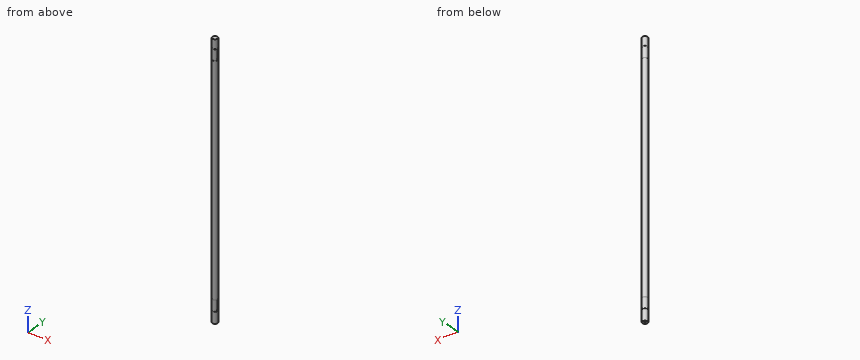
from build123d import *

# Parameters (mm, degrees)
SKETCH_2_R             = 15
EXTRUDE_1_DEPTH        = 1500
CUT_EXTRUDE_1_DEPTH    = 1501.283306579
SKETCH_4_W             = 1.6
SKETCH_4_H             = 0.7
PATTERN_LINEAR_1_COUNT = 2
PATTERN_LINEAR_1_PITCH = 1322
HOLE_WIZARD_M8_1_D     = 6.8
HOLE_WIZARD_M8_1_DEPTH = 19.75
HOLE_WIZARD_M8_1_TIP   = 2.042926105


with BuildPart() as part:
    # 草图2 → 凸台-拉伸1 (new body)
    with BuildSketch(Plane.XY):
        Circle(SKETCH_2_R)
    extrude(amount=EXTRUDE_1_DEPTH)

    # 草图3 → 切除-拉伸1 (cut, through all)
    with BuildSketch(Plane(origin=(10, 0, 0), x_dir=(0, 0, -1), z_dir=(1, 0, 0))):
        with BuildLine():
            Line((-1440, 5), (-1395, 5))
            ThreePointArc((-1395, 5), (-1390, 0), (-1395, -5))
            Line((-1395, -5), (-1440, -5))
            ThreePointArc((-1440, -5), (-1445, 0), (-1440, 5))
        make_face()
        with BuildLine():
            Line((-73, -5), (-118, -5))
            ThreePointArc((-118, -5), (-123, 0), (-118, 5))
            Line((-118, 5), (-73, 5))
            ThreePointArc((-73, 5), (-68, 0), (-73, -5))
        make_face()
    extrude(amount=CUT_EXTRUDE_1_DEPTH, mode=Mode.SUBTRACT)

    # 草图4 → 切除-旋转5 (revolve, cut)
    with BuildSketch(Plane(origin=(0, 0, 0), x_dir=(0, 0, -1), z_dir=(1, 0, 0))):
        with Locations((-1448.3, 14.65)):
            Rectangle(SKETCH_4_W, SKETCH_4_H)
        with Locations((-1386.7, 14.65)):
            Rectangle(SKETCH_4_W, SKETCH_4_H)
    cut_revolve_5 = revolve(axis=Axis((0, 0, 1445), (0, 0, 1)), mode=Mode.SUBTRACT)

    # 阵列(线性)1: 切除-旋转5 ×2
    with Locations(*[(0, 0, -i * PATTERN_LINEAR_1_PITCH) for i in range(1, PATTERN_LINEAR_1_COUNT)]):
        add(cut_revolve_5, mode=Mode.SUBTRACT)

    # M8 螺纹孔1
    with Locations(Plane(origin=(0, 0, 0), x_dir=(-1, 0, 0), z_dir=(0, 0, -1))):
        with Locations((0, 0)):
            Hole(HOLE_WIZARD_M8_1_D / 2, depth=HOLE_WIZARD_M8_1_DEPTH)
            with Locations((0, 0, -(HOLE_WIZARD_M8_1_DEPTH + HOLE_WIZARD_M8_1_TIP / 2))):  # 118° drill point
                Cone(0, HOLE_WIZARD_M8_1_D / 2, HOLE_WIZARD_M8_1_TIP, mode=Mode.SUBTRACT)


solid = part.part
Can you work these out from the model? Positions are in its coordinate system, mm. Give positions to 0.01 mm unless a question says otherwise; leave off trailing zeros. Loops run counter-clockwise (first coordinate to the right, second up) from the corner with the lowest first, then second, coordinate; pieces in that order, holes last. Notation, with made-up numbers: (34, -37) - (78, -37) arc R22 cw to (78, -22) - close; hole circle Ø7 at (53, 78.5). An arc over 180 degrees is marked (long way). Return JSON: item names as keys, results as strings.
1. I want a section at A-A on z = 980.5. Please give me the cut outline in (x, y).
Output values:
{"outline": "circle Ø30 at (0, 0)"}
2. I'm going to push flat-ended pins straight in: pin 1 Ø10 at (x, z) = (3, 572) entering from +Y; pin 2 Ø10 at (x, z) = (12, 508) entering from +Y; pin 3 Ø3 at (x, z) = (5, 1209) entering from -Y; pin 4 Ø4 at (y, z) = (6.5, 412) entering from +X. Where does each tip first touch, or does it pass through?
Output values:
{"pin 1": "stops at y = 15", "pin 2": "stops at y = 13.27", "pin 3": "stops at y = -14.59", "pin 4": "stops at x = 14.31"}
3. If I drill on line 1 (Z direction, x = 13.5, y = 0.5); line 2 (Y direction, x = 0, z = 6.5), over which ranges is the centre line in solid material (lowest first)?
Output values:
{"line 1": "z = 0 to 68.03, 122.97 to 1390.03, 1444.97 to 1500", "line 2": "y = -15 to -3.4, 3.4 to 15"}
